Read the model definition and answer for the solid it produces. Units are mm, in the model's axes. Coordinates: 2 decimals unless noted, no trailing zeros. Write each loop counter-clockwise with the first axis right and the second up, starting at its lowest first coordinate (ties: lowest second). Pieces come first, ordered by that corner, then holes.
(1) Straight lines are drawn through the part: line 1 along Y through (x, z) = (0, 3.25); line 2 along Y through (x, z) = (-65.5, 3.25); line 3 along X through (y, z) = (-103.5, -4). For each, find the intervals that lie inside material, in ascending order.
(2) The part is cut by section B-B, the plane y = 40. Determine the outline of the cut face in (x, z), and give its area (3 significant figures).
(3) The part is cut by section C-C, the plane z = 3. Determine the outline of the cut face in (x, y).
(4) The part is cut by section A-A, the plane x = 0. Determine the outline of the cut face in (y, z).
(5) The part is cut by section D-D, the plane y = -117. Determine the outline of the cut face in (x, z), and give its area (3 significant figures).
(6) Given pin 1 (5 mm diameter, centred on y = -101, z = 0, fed in from +X); pin 2 (24 mm diameter, centred on x = 0, y = -110, fed in from +Z); pin 3 (3 mm diameter, centred on x = -90.5, z = 2.5, fed in from -Y), each flat-ended and moving along its own axis, determine where each tip first touches the part or whether it passes through.
```python
from build123d import *

# Parameters (mm, degrees)
SKETCH1_R           = 15
SKETCH1_R_2         = 12.5
BOSS_EXTRUDE1_DEPTH = 5
FILLET1_R           = 20


with BuildPart() as part:
    # Sketch1 → Boss-Extrude1 (new, symmetric)
    # profile 1 of 3: a face of its own
    with BuildSketch(Plane.XY):
        with BuildLine():
            Line((30, -110), (30, -75))
            Line((30, -75), (-30, -75))
            Line((-30, -75), (-30, -110))
            ThreePointArc((-30, -110), (0, -140), (30, -110))
        make_face()
        with Locations((0, -110)):
            Circle(SKETCH1_R, mode=Mode.SUBTRACT)
    # profile 2 of 3: a face of its own
    with BuildSketch(Plane.XY):
        with BuildLine():
            Line((30, -75), (110, -75))
            Line((110, -75), (110, 75))
            Line((110, 75), (-110, 75))
            Line((-110, 75), (-110, -75))
            Line((-110, -75), (-30, -75))
            ThreePointArc((-30, -75), (0, -45), (30, -75))
        make_face()
        with Locations((0, 40)):
            Circle(SKETCH1_R_2, mode=Mode.SUBTRACT)
    # profile 3 of 3: a face of its own
    with BuildSketch(Plane.XY):
        with BuildLine():
            Line((-30, -75), (30, -75))
            ThreePointArc((30, -75), (0, -45), (-30, -75))
        make_face()
    extrude(amount=BOSS_EXTRUDE1_DEPTH, both=True)

    # Fillet1
    fillet1_edges = [part.edges().sort_by_distance(p)[0] for p in [
        (-30, -75, 0),
        (30, -75, 0),
    ]]
    fillet(fillet1_edges, radius=FILLET1_R)


solid = part.part
```
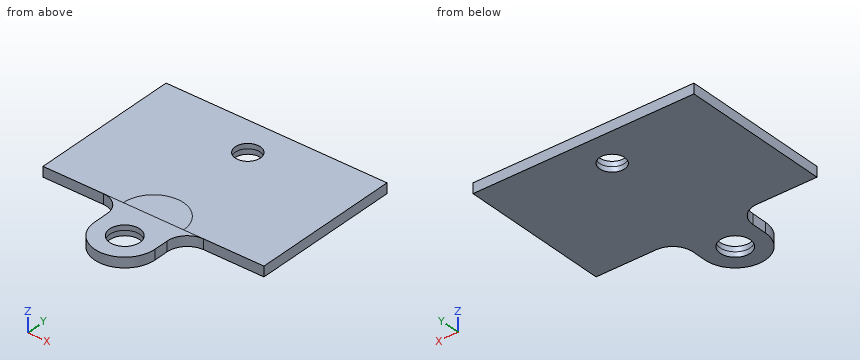
Computed:
1. line 1: y = -140 to -125, -95 to 27.5, 52.5 to 75
1. line 2: y = -75 to 75
1. line 3: x = -30 to -13.52, 13.52 to 30
2. outline: (-110, -5) - (-12.5, -5) - (-12.5, 5) - (-110, 5) - close; (12.5, -5) - (110, -5) - (110, 5) - (12.5, 5) - close
2. area: 1,950 mm2
3. outline: (-110, -75) - (-50, -75) arc R20 cw to (-30, -95) - (-30, -110) arc R30 ccw to (30, -110) - (30, -95) arc R20 cw to (50, -75) - (110, -75) - (110, 75) - (-110, 75) - close; hole circle Ø30 at (0, -110); hole circle Ø25 at (0, 40)
4. outline: (-140, -5) - (-125, -5) - (-125, 5) - (-140, 5) - close; (-95, -5) - (27.5, -5) - (27.5, 5) - (-95, 5) - close; (52.5, -5) - (75, -5) - (75, 5) - (52.5, 5) - close
5. outline: (-29.17, -5) - (-13.27, -5) - (-13.27, 5) - (-29.17, 5) - close; (13.27, -5) - (29.17, -5) - (29.17, 5) - (13.27, 5) - close
5. area: 318 mm2
6. pin 1: stops at x = 30
6. pin 2: passes through
6. pin 3: stops at y = -75
